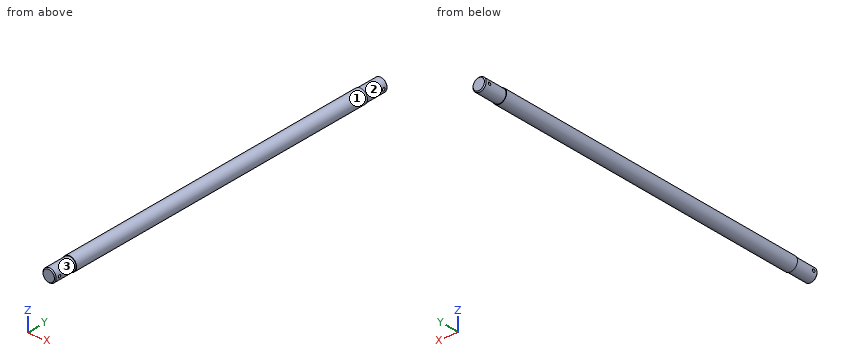
from build123d import *

# Parameters (mm, degrees)
CHAMFER1_SIZE           = 1
CUT_EXTRUDE1_DEPTH      = 401.140600289
CUT_EXTRUDE1_DEPTH_BACK = 401.140600289
SKETCH3_R               = 1.5


with BuildPart() as part:
    # Sketch1 → Revolve1 (revolve)
    with BuildSketch(Plane.XY, mode=Mode.PRIVATE) as revolve1_sk:
        Polygon((0, 0), (7, 0), (7, 25), (7.5, 25), (7.5, 375), (7, 375), (7, 400), (0, 400), align=None)
    revolve(revolve1_sk.sketch.rotate(Axis((0, 0, 0), (0, -1, 0)), 90), axis=Axis((0, 0, 0), (0, -1, 0)))

    # Chamfer1
    chamfer1_edges = [part.edges().sort_by_distance(p)[0] for p in [
        (0, 400, -7),
        (0, 0, -7),
    ]]
    chamfer(chamfer1_edges, length=CHAMFER1_SIZE)

    # Sketch3 → Cut-Extrude1 (cut, two sides: drawn at the far end of the back side and taken through both)
    with BuildSketch(Plane(origin=(0, 0, 0), x_dir=(0, 0, -1), z_dir=(1, 0, 0)).offset(-CUT_EXTRUDE1_DEPTH_BACK)):
        with Locations((0, 395)):
            Circle(SKETCH3_R)
        with Locations((0, 5)):
            Circle(SKETCH3_R)
    extrude(amount=CUT_EXTRUDE1_DEPTH + CUT_EXTRUDE1_DEPTH_BACK, mode=Mode.SUBTRACT)


solid = part.part
Work out the finished part from the listing and answer in its coordinate system (mm). Face numbers are marked on the shaded views. A direction names the side the tool comes from. Round coordinates to 2 decimals unless told otherwise and drop trailing zeros. Write each loop counter-clockwise with the first axis right and the second up, starting at its lowest first coordinate (ties: lowest second). Pieces come first, ordered by that corner, then holes. Notation, with made-up numbers: (44, -18.75) - (98, -18.75) arc R22 ccw to (98, 3.25) - close; hole circle Ø2 at (29, -19.5). An arc over 180 degrees is marked (long way). Answer in a Markdown table with one row per item. Add a question column.
1. Given pin 1 (6 mm diameter, centred on y = 104.5, z = 5, fed in from -X); pin 2 (4 mm diameter, centred on y = 395, z = 0, fed in from +X); pin 3 (3 mm diameter, centred on y = 94, z = -3, fed in from +X), each flat-ended and moving along its own axis, determine where each tip first touches the part or whether it passes through.
2. For the marked faces 1, 2 and 3, determine the directions among +Z, -Z, +X, -X, +Y, -Y from which every point of the face is accessible in a straight line to the end or side of a thin tool.
3. Find the intervals of material crossed by line 1 along Y through (x, z) = (0.25, 0); line 2 along Y through (x, z) = (5.75, -1); line 3 along Z through (x, y) = (-3.25, 5), in increasing order. Write a range as from..to.
4. A cutting plane is placed at A-A, the plane y = 371.5. Determine the outline of the cut face in (x, z).
5. A cutting plane is placed at B-B, the plane x = -3.25. Count the separate pieces of the cut face and the enclosed holes in it, and give its area (3 significant figures).
Worked out:
| question | item | result |
|---|---|---|
| 1 | pin 1 | x = -7.23 |
| 1 | pin 2 | x = 7 |
| 1 | pin 3 | x = 7.35 |
| 2 | face 1 | +Y, -Y |
| 2 | face 2 | +Y |
| 2 | face 3 | -Y |
| 3 | line 1 | 0..3.5, 6.5..393.5, 396.5..400 |
| 3 | line 2 | 0..3.88, 6.12..393.88, 396.12..400 |
| 3 | line 3 | -6.2..-1.5, 1.5..6.2 |
| 4 | outline | circle Ø15 at (0, 0) |
| 5 | separate pieces | 1 |
| 5 | enclosed holes | 2 |
| 5 | area | 5,340 mm^2 |
